Source: CAD feature listing. Evaluate the final solid. Frame: model axes, mm. Give positions to 0.01 mm unless a question says otherwise; leave off trailing zeros. Order: outer loops, then holes, each group sorted by start corner. A loop starts at its lowest first (then second) coordinate and runs counter-clockwise, first axis right, second up. Notation, with made-up numbers: (65, 67.5) -> (110, 67.5) arc R10 ccw to (110, 78.5) -> close; hole circle Ø6 at (31, 17). An arc over 180 degrees is marked (long way). Use CSV: the item, a comma, the result in double quotes.
```python
from build123d import *

# Parameters (mm, degrees)
CUT_EXTRUDE1_DEPTH      = 1.6
CUT_EXTRUDE1_DEPTH_BACK = 1.6
SKETCH3_W               = 14
SKETCH3_H               = 14


with BuildPart() as part:
    # Sketch1 → Revolve1 (revolve)
    with BuildSketch(Plane.XY, mode=Mode.PRIVATE) as revolve1_sk:
        with BuildLine():
            Line((-1.6, 0), (-1.6, 3.48))
            ThreePointArc((-1.6, 3.48), (-1.389116882, 3.989116882), (-0.88, 4.2))
            Line((-0.88, 4.2), (1.6, 4.2))
            Line((1.6, 4.2), (1.6, 0))
            Line((1.6, 0), (-1.6, 0))
        make_face()
    revolve(revolve1_sk.sketch.rotate(Axis((1.6, 0, 0), (-1, 0, 0)), 270), axis=Axis((1.6, 0, 0), (-1, 0, 0)))

    # Sketch2 → Cut-Revolve1 (revolve, cut)
    with BuildSketch(Plane.XY, mode=Mode.PRIVATE) as cut_revolve1_sk:
        Polygon((-1.6, 0), (-1.6, 2), (-1.221, 1.621), (1.221, 1.621), (1.6, 2), (1.6, 0), align=None)
    revolve(cut_revolve1_sk.sketch.rotate(Axis((1.6, 0, 0), (-1, 0, 0)), 270), axis=Axis((1.6, 0, 0), (-1, 0, 0)), mode=Mode.SUBTRACT)

    # Sketch3 → Cut-Extrude1 (cut, two sides: drawn at the far end of the back side and taken through both)
    with BuildSketch(Plane(origin=(0, 0, 0), x_dir=(0, 0, -1), z_dir=(1, 0, 0)).offset(-CUT_EXTRUDE1_DEPTH_BACK)):
        Rectangle(SKETCH3_W, SKETCH3_H)
        Polygon((-3.5, 2.020725942), (-3.5, -2.020725942), (0, -4.041451884), (3.5, -2.020725942), (3.5, 2.020725942), (0, 4.041451884), align=None, mode=Mode.SUBTRACT)
    extrude(amount=CUT_EXTRUDE1_DEPTH + CUT_EXTRUDE1_DEPTH_BACK, mode=Mode.SUBTRACT)


solid = part.part
```
1. Section query A-A on x = -0.8. Return loops of the section in (y, z).
Answer below:
outline,"(-4.04, 0) -> (-2.02, -3.5) -> (2.02, -3.5) -> (4.04, 0) -> (2.02, 3.5) -> (-2.02, 3.5) -> close; hole circle Ø3.24 at (0, 0)"
2. Pin query (flat end, axial travel): P1, Ø1, axis at x = 1.5, z = 2, coming from the -Y side; P2, Ø1.9, axis at y = 0, z = 0, coming from the +X side; P3, Ø1.5, axis at x = 0.5, z = 2, coming from the -Y side. Return the tip coordinate at first contact, or that it passes through.
Answer below:
P1,"stops at y = -3.18"
P2,"passes through"
P3,"stops at y = -3.32"
3. Mould query, pull axis Z, two halves, no side actions, for faces 1 (the flat face through (0, 0, 3.5)), 2 (the flat face through (0, 3, -1.8)), 3 (the cylindrical face through (0.017, -1.438, 0.748)). Classes: released by +Z, released by -Z, zero draft, split by the parting line, or undercut.
Answer below:
face 1,"released by +Z"
face 2,"released by -Z"
face 3,"undercut"
4. Ray query, line 1 along Y through (x, z) = (-1.1, -0.25); line 2 along X through (y, z) = (0.5, 1.75); line 3 along Y through (x, z) = (1.35, -1.25). Return the intervals inside material, ascending.
Answer below:
line 1,"y = -3.9 to -1.6, 1.6 to 3.9"
line 2,"x = -1.42 to 1.42"
line 3,"y = -3.32 to -1.22, 1.22 to 3.32"
